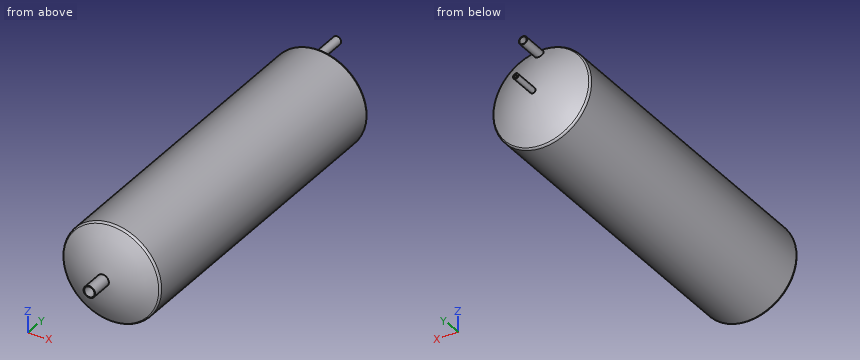
```python
from build123d import *

# Parameters (mm, degrees)
BOSS_EXTRUDE1_REACH      = 1349.915
BOSS_EXTRUDE1_END_RADIUS = 331.651906797
SKETCH2_R                = 21
SKETCH2_R_2              = 18.5
SKETCH3_R                = 18.5
CUT_EXTRUDE1_DEPTH       = 526
BOSS_EXTRUDE3_REACH      = 1443.406
BOSS_EXTRUDE3_END_RADIUS = 331.651906797
SKETCH5_R                = 10
SKETCH5_R_2              = 5
SKETCH6_R                = 5
CUT_EXTRUDE2_DEPTH       = 190
BOSS_EXTRUDE5_REACH      = 1404.016
BOSS_EXTRUDE5_END_RADIUS = 331.651906797
SKETCH8_R                = 15
SKETCH8_R_2              = 13
SKETCH9_R                = 13.000001432
CUT_EXTRUDE3_DEPTH       = 107


with BuildPart() as part:
    # Sketch1 → Revolve1 (revolve)
    with BuildSketch(Plane.XY, mode=Mode.PRIVATE) as revolve1_sk:
        with BuildLine():
            Line((175, -569.454864482), (175, 569.454864482))
            ThreePointArc((175, 569.454864482), (173.697634466, 574.389553398), (170.129769061, 578.03888856))
            ThreePointArc((170.129769061, 578.03888856), (88.246082503, 613.044224248), (0, 625))
            Line((0, 625), (0, 620))
            ThreePointArc((0, 620), (85.508108026, 608.609622217), (165.052867094, 575.232855612))
            ThreePointArc((165.052867094, 575.232855612), (168.67550203, 571.57683653), (170, 566.603340322))
            Line((170, 566.603340322), (170, -566.603340322))
            ThreePointArc((170, -566.603340322), (168.67550203, -571.57683653), (165.052867094, -575.232855612))
            ThreePointArc((165.052867094, -575.232855612), (85.508108026, -608.609622217), (0, -620))
            Line((0, -620), (0, -625))
            ThreePointArc((0, -625), (88.246082503, -613.044224248), (170.129769061, -578.03888856))
            ThreePointArc((170.129769061, -578.03888856), (173.697634466, -574.389553398), (175, -569.454864482))
        make_face()
    revolve(revolve1_sk.sketch.rotate(Axis((0, 0, 0), (0, 1, 0)), 90), axis=Axis((0, 0, 0), (0, 1, 0)))

    # Boss-Extrude1: up to this sphere (the profile starts outside it)
    boss_extrude1_end = Location((0, -293.348093203, 0)) * Sphere(BOSS_EXTRUDE1_END_RADIUS, mode=Mode.PRIVATE)
    # Sketch2 → Boss-Extrude1 (add, up to the surface)
    with BuildSketch(Plane(origin=(0, -700, 0), x_dir=(1, 0, 0), z_dir=(0, 1, 0)), mode=Mode.PRIVATE) as boss_extrude1_sk1:
        with Locations(Location((0, 0, 0), (0, 0, 180))):
            Circle(SKETCH2_R)
        with Locations(Location((0, 0, 0), (0, 0, 270))):
            Circle(SKETCH2_R_2, mode=Mode.SUBTRACT)
    boss_extrude1_tool1 = extrude(boss_extrude1_sk1.sketch, amount=BOSS_EXTRUDE1_REACH, mode=Mode.PRIVATE) - boss_extrude1_end
    add(boss_extrude1_tool1.solids().sort_by_distance((20.40603, -700, 0))[0])

    # Sketch3 → Cut-Extrude1 (cut)
    with BuildSketch(Plane(origin=(0, -700, 0), x_dir=(1, 0, 0), z_dir=(0, 1, 0))):
        Circle(SKETCH3_R)
    extrude(amount=CUT_EXTRUDE1_DEPTH, mode=Mode.SUBTRACT)

    # Boss-Extrude3: up to this sphere (the profile starts outside it)
    boss_extrude3_end = Location((0, 293.348093203, 0)) * Sphere(BOSS_EXTRUDE3_END_RADIUS, mode=Mode.PRIVATE)
    # Sketch5 → Boss-Extrude3 (add, up to the surface)
    with BuildSketch(Plane(origin=(0, 720, 0), x_dir=(1, 0, 0), z_dir=(0, 1, 0)), mode=Mode.PRIVATE) as boss_extrude3_sk1:
        with Locations(Location((0, 0, 0), (0, 0, 270))):
            Circle(SKETCH5_R)
        with Locations(Location((0, 0, 0), (0, 0, 270))):
            Circle(SKETCH5_R_2, mode=Mode.SUBTRACT)
    boss_extrude3_tool1 = extrude(boss_extrude3_sk1.sketch, amount=-BOSS_EXTRUDE3_REACH, mode=Mode.PRIVATE) - boss_extrude3_end
    add(boss_extrude3_tool1.solids().sort_by_distance((0, 720, -9.717157))[0])

    # Sketch6 → Cut-Extrude2 (cut)
    with BuildSketch(Plane(origin=(0, 720, 0), x_dir=(1, 0, 0), z_dir=(0, 1, 0))):
        with Locations(Location((0, 0, 0), (0, 0, 270))):
            Circle(SKETCH6_R)
    extrude(amount=-CUT_EXTRUDE2_DEPTH, mode=Mode.SUBTRACT)

    # Boss-Extrude5: up to this sphere (the profile starts outside it)
    boss_extrude5_end = Location((0, 293.348093203, 0)) * Sphere(BOSS_EXTRUDE5_END_RADIUS, mode=Mode.PRIVATE)
    # Sketch8 → Boss-Extrude5 (add, up to the surface)
    with BuildSketch(Plane(origin=(0, 680, 0), x_dir=(1, 0, 0), z_dir=(0, 1, 0)), mode=Mode.PRIVATE) as boss_extrude5_sk1:
        with Locations(Location((0, -150, 0), (0, 0, 270.000000007))):
            Circle(SKETCH8_R)
        with Locations(Location((0, -150, 0), (0, 0, 270))):
            Circle(SKETCH8_R_2, mode=Mode.SUBTRACT)
    boss_extrude5_tool1 = extrude(boss_extrude5_sk1.sketch, amount=-BOSS_EXTRUDE5_REACH, mode=Mode.PRIVATE) - boss_extrude5_end
    add(boss_extrude5_tool1.solids().sort_by_distance((0, 680, 135.424264))[0])

    # Sketch9 → Cut-Extrude3 (cut)
    with BuildSketch(Plane(origin=(0, 680, 0), x_dir=(1, 0, 0), z_dir=(0, 1, 0))):
        with Locations(Location((0, -150, 0), (0, 0, 270))):
            Circle(SKETCH9_R)
    extrude(amount=-CUT_EXTRUDE3_DEPTH, mode=Mode.SUBTRACT)


solid = part.part
```
Can you work these out from the model? Positions are in its coordinate system, mm. Coordinates: 2 decimals unless noted, no trailing zeros. Order: outer loops, then holes, each group sorted by start corner. A loop starts at its lowest first (then second) coordinate and runs counter-clockwise, first axis right, second up. Notation, with made-up numbers: (31.5, -26.75) -> (49.5, -26.75) arc R20 cw to (49.5, 11.25) -> close; hole circle Ø6 at (-39, 67.25). An arc over 180 degrees is marked (long way). Write each question's results on one line, items separated by ' | '.
Item 1: I want a section at A-A, the plane y = 186. Write out the boundary of the cut face in (x, z), then the cut area to 3 significant figures.
Results are:
outline: circle Ø350 at (0, 0); hole circle Ø340 at (0, 0) | area: 5,420 mm²
Item 2: I'm going to push flat-ended pins straight in: pin 1 Ø1.5 at (y, z) = (279, 86) entering from -X; pin 2 Ø5 at (x, y) = (136.5, -366.5) entering from +Z; pin 3 Ø8 at (y, z) = (-454.5, 127.5) entering from -X; pin 4 Ø6 at (x, z) = (0, 0) entering from -Y. Where does each tip first touch, or does it pass through?
Results are:
pin 1: x = -152.83 | pin 2: z = 112.56 | pin 3: x = -123.99 | pin 4: through
Item 3: If I drill on line 1 along X through (y, z) = (-100, 0); line 2 along X through (y, z) = (642, 0); line 3 along Z through (x, y) = (-114.5, 141.5), over which ranges is the centre line in solid material (lowest first)?
Results are:
line 1: -175 to -170, 170 to 175 | line 2: -10 to -5, 5 to 10 | line 3: -132.34 to -125.66, 125.66 to 132.34
